from build123d import *

# Parameters (mm, degrees)
SKETCH_1_W                    = 360
SKETCH_1_H                    = 250
EXTRUDE_1_DEPTH               = 20
HOLE_WIZARD_M10_1_D           = 12
HOLE_WIZARD_M10_1_CBORE_D     = 18
HOLE_WIZARD_M10_1_CBORE_DEPTH = 10.6
HOLE_WIZARD_M52_1_D           = 61
HOLE_WIZARD_M12_1_D           = 15
HOLE_WIZARD_M12_1_CBORE_D     = 20
HOLE_WIZARD_M12_1_CBORE_DEPTH = 12.6
CHAMFER_1_SIZE                = 1
CHAMFER_2_SIZE                = 5


with BuildPart() as part:
    # 草图1 → 凸台-拉伸1 (new body)
    with BuildSketch(Plane.XZ.offset(-63)):
        with Locations((315.1, -245)):
            Rectangle(SKETCH_1_W, SKETCH_1_H)
    extrude(amount=-EXTRUDE_1_DEPTH)

    # M10 六角凹头螺钉的柱形沉头孔1 (through all)
    with Locations(Plane(origin=(0, 83, 0), x_dir=(-1, 0, 0), z_dir=(0, 1, 0))):
        with Locations((-470.1, -345), (-430.1, -345), (-470.1, -145), (-430.1, -145), (-200.1, -145), (-200.1, -345), (-160.1, -145), (-160.1, -345)):
            CounterBoreHole(HOLE_WIZARD_M10_1_D / 2, HOLE_WIZARD_M10_1_CBORE_D / 2, HOLE_WIZARD_M10_1_CBORE_DEPTH)

    # M52 间隙孔1 (through all)
    with Locations(Plane(origin=(0, 63, 0), x_dir=(-1, 0, 0), z_dir=(0, -1, 0))):
        with Locations((-315.1, 245)):
            Hole(HOLE_WIZARD_M52_1_D / 2)

    # M12 六角凹头螺钉的柱形沉头孔1 (through all)
    with Locations(Plane(origin=(0, 63, 0), x_dir=(-1, 0, 0), z_dir=(0, -1, 0))):
        with Locations((-245.817967697, 205), (-275.1, 175.717967697), (-315.1, 165), (-355.1, 175.717967697), (-384.382032303, 205), (-395.1, 245), (-384.382032303, 285), (-355.1, 314.282032303), (-315.1, 325), (-275.1, 314.282032303), (-245.817967697, 285), (-235.1, 245)):
            CounterBoreHole(HOLE_WIZARD_M12_1_D / 2, HOLE_WIZARD_M12_1_CBORE_D / 2, HOLE_WIZARD_M12_1_CBORE_DEPTH)

    # 倒角1
    chamfer_1_edges = [part.edges().sort_by_distance(p)[0] for p in [
        (284.6, 63, -245),
    ]]
    chamfer(chamfer_1_edges, length=CHAMFER_1_SIZE)

    # 倒角2
    chamfer_2_edges = [part.edges().sort_by_distance(p)[0] for p in [
        (495.1, 73, -120),
        (495.1, 73, -370),
        (135.1, 73, -370),
        (135.1, 73, -120),
    ]]
    chamfer(chamfer_2_edges, length=CHAMFER_2_SIZE)


solid = part.part
Can you work these out from the model? Positions are in its coordinate system, mm. A direction names the side the tool comes from. Round coordinates to 2 decimals unless told otherwise and drop trailing zeros. Order: outer loops, then holes, each group sorted by start corner. A loop starts at its lowest first (then second) coordinate and runs counter-clockwise, first axis right, second up. Notation, with made-up numbers: (55.25, 71.25) - (64.25, 71.25) arc R22 cw to (64.25, 98.25) - close; hole circle Ø5 at (-28.75, 4). An arc over 180 degrees is marked (long way). Answer in a Markdown table with one row per item.
(1) Suppose I cut it at C-C, the plane z = -245. Please give me the cut outline in (x, y).
From the geometry:
| item | result |
|---|---|
| outline | (135.1, 63) - (225.1, 63) - (225.1, 75.6) - (227.6, 75.6) - (227.6, 83) - (135.1, 83) - close; (242.6, 75.6) - (245.1, 75.6) - (245.1, 63) - (283.6, 63) - (284.6, 64) - (284.6, 83) - (242.6, 83) - close; (345.6, 64) - (346.6, 63) - (385.1, 63) - (385.1, 75.6) - (387.6, 75.6) - (387.6, 83) - (345.6, 83) - close; (402.6, 75.6) - (405.1, 75.6) - (405.1, 63) - (495.1, 63) - (495.1, 83) - (402.6, 83) - close |
(2) For P1, Ø16, axis at x = 355.1, z = -175.72, coming from the -Y side, with a flat end and sliding along its axis, tell me the tip position at first contact or that it passes through.
From the geometry:
| item | result |
|---|---|
| P1 | stops at y = 75.6 |
(3) Please list where these lines run through material, in increasing order: L1, parallel to Z at x = 355.1, y = 68.25; L2, parallel to X at y = 71.75, z = -205; L3, parallel to X at y = 67, z = -345. Write a range as from..to.
From the geometry:
| item | result |
|---|---|
| L1 | z = -370..-324.28, -304.28..-185.72, -165.72..-120 |
| L2 | x = 135.1..235.82, 255.82..374.38, 394.38..495.1 |
| L3 | x = 135.1..154.1, 166.1..194.1, 206.1..424.1, 436.1..464.1, 476.1..495.1 |
(4) Suppose I cut it at B-B, the plane x = 430.1. Please give me the cut outline in (y, z).
From the geometry:
| item | result |
|---|---|
| outline | (63, -370) - (83, -370) - (83, -354) - (72.4, -354) - (72.4, -351) - (63, -351) - close; (63, -339) - (72.4, -339) - (72.4, -336) - (83, -336) - (83, -154) - (72.4, -154) - (72.4, -151) - (63, -151) - close; (63, -139) - (72.4, -139) - (72.4, -136) - (83, -136) - (83, -120) - (63, -120) - close |
(5) Which directions (+Z, -Z, +X, -X, +Y, -Y) give clear straight access to the entire face, cutting with the end or side of a thin tool? Please do faces 3 (the face through (242.03, 79.35, -242.13)), 4 (the face through (385.56, 69.21, -248)), 5 (the face through (202.051, 77.774, -353.786)).
From the geometry:
| item | result |
|---|---|
| face 3 | +Y, -Y |
| face 4 | -Y |
| face 5 | +Y |
(6) If we mould it in two halves opening along X, with no side actions, what happens to faces 1 (the face through (282.03, 79.35, -172.85)), 2 (the face through (313, 73, -370))? For each: released by +X, released by -X, zero draft, split by the parting line, or undercut.
From the geometry:
| item | result |
|---|---|
| face 1 | undercut |
| face 2 | zero draft |
(7) Suppose I cut it at A-A, the plane z = -285. Please give me the cut outline in (x, y).
From the geometry:
| item | result |
|---|---|
| outline | (135.1, 63) - (235.82, 63) - (235.82, 75.6) - (238.32, 75.6) - (238.32, 83) - (135.1, 83) - close; (253.32, 75.6) - (255.82, 75.6) - (255.82, 63) - (374.38, 63) - (374.38, 75.6) - (376.88, 75.6) - (376.88, 83) - (253.32, 83) - close; (391.88, 75.6) - (394.38, 75.6) - (394.38, 63) - (495.1, 63) - (495.1, 83) - (391.88, 83) - close |
